Source: CAD feature listing. Evaluate the final solid. Frame: model axes, mm. A direction names the side the tool comes from. Round coordinates to 2 decimals unless told otherwise and drop trailing zeros. Write item = value, one per line. Start each with the question number.
(1) Ray query, line 1 (Y direction, x = -5.4, z = 0.1); line 2 (X direction, y = -1.5, z = 1.7); line 3 (Y direction, x = -5.4, z = 0.7). Return the intervals inside material, ascending.
(2) Draft query along Y for faces 1 (the face through (-7.5, 0.1, 0)), 2 (the face through (17.7, 2.5, 0.1)), 3 (the face through (39.297, -1.745, -0.03)). Return one class per face: released by +Y, released by -Y, zero draft, split by the parting line, or undercut.
(3) Reachability of faces 4 (the face through (39.12, -0.64, -0.03)), 5 (the face through (20.3, -2.5, 0.1)) from +Z, -Z, +X, -X, +Y, -Y: full face, straight path, thin tool, end or side. Return the list, or none.
(4) Contact query for flat-ended pins moving along their axis: pin 1 Ø1 at (x, z) = (18.5, -1) entering from -Y; pin 2 Ø2 at (x, z) = (-1.5, -1) entering from -Y; pin 3 Ø3 at (x, y) = (23, 1) entering from +Z. Output: stop coordinate, or through.
from build123d import *

# Parameters (mm, degrees)
CONECUT_DEPTH      = 41.341170006
CONECUT_DEPTH_BACK = 41.341170006


with BuildPart() as part:
    # Body: sweep along a path in Sketch2
    with BuildLine(Plane.XY) as body_path:
        Line((36, 2.5), (0, 2.5))
        ThreePointArc((0, 2.5), (-1.229728386, 2.730698436), (-2.292225201, 3.391420912))
        ThreePointArc((-2.292225201, 3.391420912), (-10, 0), (-2.292225201, -3.391420912))
        ThreePointArc((-2.292225201, -3.391420912), (-1.229728386, -2.730698436), (0, -2.5))
        Line((0, -2.5), (40, -2.5))
    # Sketch1 → Body (sweep)
    with BuildSketch(Plane(origin=(36, 0, 0), x_dir=(0, 0, -1), z_dir=(1, 0, 0))):
        with BuildLine():
            Line((-2.4999992, 0.002), (2.4999992, 0.002))
            ThreePointArc((2.4999992, 0.002), (0, 2.5), (-2.4999992, 0.002))
        make_face()
    sweep(path=body_path.line)

    # Sketch3 → ConeCut (cut, two sides: drawn at the far end of the back side and taken through both)
    with BuildSketch(Plane.XY.offset(-CONECUT_DEPTH_BACK)):
        Polygon((36, 1.251), (34.210475082, 2.51), (40.01, 2.51), (40.01, -2.51), (38.210475082, -2.51), (40, -1.251), (38.204873421, 0), (34.204873421, 0), align=None)
    extrude(amount=CONECUT_DEPTH + CONECUT_DEPTH_BACK, mode=Mode.SUBTRACT)


solid = part.part
Evaluation:
q1.line_1 = -4.6 to -2.1, 2.1 to 4.6
q1.line_2 = -9.04 to -6.87, -3.92 to 39.65
q1.line_3 = -4.5 to -2.1, 2.1 to 4.5
q2.face_1 = undercut
q2.face_2 = released by +Y
q2.face_3 = released by -Y
q3.face_4 = +Z, -Z, +X, +Y
q3.face_5 = +X, -Y
q4.pin_1 = -2.45
q4.pin_2 = -3.41
q4.pin_3 = 2.5
